from build123d import *

# Parameters (mm, degrees)
SKETCH2_R          = 17
CUT_EXTRUDE1_DEPTH = 70
CHAMFER1_SIZE      = 1
SKETCH7_W          = 8
SKETCH7_H          = 8
CUT_EXTRUDE2_DEPTH = 70


with BuildPart() as part:
    # Sketch1 → Revolve1 (revolve)
    with BuildSketch(Plane.XY):
        Polygon((0, 0), (0, 50), (3, 50), (7.003672577, 39), (15.996327423, 39), (20, 50), (22, 50), (26.003672577, 39), (34.996327423, 39), (39, 50), (42, 50), (42, 30), (54, 30), (54, 0), align=None)
    revolve(axis=Axis((54, 0, 0), (-1, 0, 0)))

    # Sketch2 → Cut-Extrude1 (cut)
    with BuildSketch(Plane(origin=(54, 0, 0), x_dir=(0, 0, -1), z_dir=(1, 0, 0))):
        with Locations(Location((0, 0, 0), (0, 0, 90))):
            Circle(SKETCH2_R)
    extrude(amount=-CUT_EXTRUDE1_DEPTH, mode=Mode.SUBTRACT)

    # Sketch5 → M6 Tapped Hole1 (revolve, cut)
    with BuildSketch(Plane.YZ.offset(46.5)):
        Polygon((0, 0), (0, 51.502151548), (2.5, 50), (2.5, 0), align=None)
    revolve(axis=Axis((46.5, 0, -6.35), (0, 0, 1)), mode=Mode.SUBTRACT)

    # Chamfer1
    chamfer1_edges = [part.edges().sort_by_distance(p)[0] for p in [
        (54, -30, 0),
    ]]
    chamfer(chamfer1_edges, length=CHAMFER1_SIZE)

    # Sketch7 → Cut-Extrude2 (cut)
    with BuildSketch(Plane(origin=(54, 0, 0), x_dir=(0, 0, -1), z_dir=(1, 0, 0))):
        with Locations((-17, 0)):
            Rectangle(SKETCH7_W, SKETCH7_H)
    extrude(amount=-CUT_EXTRUDE2_DEPTH, mode=Mode.SUBTRACT)


solid = part.part
For this review, take the finished solid that the model builds, in its own axes (mm). A direction names the side the tool comes from. Coordinates: 2 decimals unless noted, no trailing zeros. Loops run counter-clockwise (first coordinate to the right, second up) from the corner with the lowest first, then second, coordinate; pieces in that order, holes last. Notation, with made-up numbers: (-12, 70) -> (43, 70) arc R26 ccw to (43, 85) -> close; hole circle Ø1 at (68, 61.25). An arc over 180 degrees is marked (long way). Write each question's results on one line, items separated by ' | '.
Q1. Mouldability with a two-part tool opening along Z and no side actions: class faces 1 (the flat face through (54, 12.5, 12.5)), 2 (the cylindrical face through (27.378, -0.691, -16.986)), 3 (the flat face through (27, 0, 21)), 4 (the cylindrical face through (21.01, 47.69, -15.02)) as +Z half, -Z half, draft (parallel to the pull), parting line (faces both ways), or undercut.
Taken from the geometry:
face 1: draft | face 2: undercut | face 3: undercut | face 4: parting line
Q2. Add section C-C, the plane x = 28. State the section outline as (y, z) points.
Taken from the geometry:
outline: circle Ø78 at (0, 0); hole (-4, 16.52) arc R17 ccw (long way) to (4, 16.52) -> (4, 21) -> (-4, 21) -> close
Q3. Add section A-A, the plane y = 0. Count the separate pieces of the cut face and the enclosed holes in it, then the cut area to 3 significant figures.
Taken from the geometry:
separate pieces: 3 | enclosed holes: 0 | area: 2,250 mm²
Q4. Add section D-D, the plane x = 46.5. State the section outline as (y, z) points, then the cut area to 3 significant figures.
Taken from the geometry:
outline: (-4, 16.52) -> (-4, 21) -> (-2.5, 21) -> (-2.5, 29.9) arc R30 ccw (long way) to (2.5, 29.9) -> (2.5, 21) -> (4, 21) -> (4, 16.52) arc R17 cw (long way) to start | area: 1,840 mm²
Q5. Machinability: for faces 5 (the flat face through (42, 22, 22)), 6 (the cylindrical face through (48.94, -0.54, 25.44)), 7 (the flat face through (27, -4, 19)), 8 (the cylindrical face through (30.563, -5.077, -38.668)), 9 (the flat face through (0, 1, 22)), which of the approach directions +Z, -Z, +X, -X, +Y, -Y give a long, thin tool a straight path to every point of the face, cutting with its end or side? Answer none if there is none.
Taken from the geometry:
face 5: +X | face 6: +Z | face 7: +X, -X | face 8: none | face 9: +Z, -Z, -X, +Y, -Y
Q6. For pin 1 Ø4 at (x, y) = (46.5, 0) entering from -Z; pin 2 Ø12 at (x, y) = (8.5, 29.5) entering from +Z; pin 3 Ø2 at (x, z) = (40.5, -21) entering from -Y, all flat-tipped, find the tip position at first contact; note any pin that passes through.
Taken from the geometry:
pin 1: z = -30 | pin 2: z = 42.02 | pin 3: y = -45.83
Q7. To check wall thickness, follow line 1 along X through (y, z) = (0, 25); line 2 along X through (y, z) = (-18, -36); line 3 along X through (y, z) = (41, 8.5). State the ranges of each line that lie inside material, in increasing order. Write a range as [from, to].
Taken from the geometry:
line 1: [0, 44], [49, 54] | line 2: [0, 6.55], [16.45, 25.55], [35.45, 42] | line 3: [0, 5.96], [17.04, 24.96], [36.04, 42]
